```python
from build123d import *

# Parameters (mm, degrees)
BOSS_EXTRUDE1_DEPTH = 12
BOSS_EXTRUDE2_DEPTH = 15
SKETCH3_R           = 5
BOSS_EXTRUDE3_DEPTH = 25
CHAMFER1_SIZE       = 0.5


with BuildPart() as part:
    # Sketch1 → Boss-Extrude1 (new body)
    with BuildSketch(Plane.XY):
        with BuildLine():
            Line((2.645751311, 3), (-2.645751311, 3))
            ThreePointArc((-2.645751311, 3), (-1.645751311, -3.645751311), (4, 0))
            ThreePointArc((4, 0), (3.645751311, 1.645751311), (2.645751311, 3))
        make_face()
    extrude(amount=-BOSS_EXTRUDE1_DEPTH)

    # Sketch2 → Boss-Extrude2 (add)
    # profile 1 of 2: a face of its own
    with BuildSketch(Plane(origin=(0, 0, -12), x_dir=(-1, 0, 0), z_dir=(0, 0, -1))):
        with BuildLine():
            Line((5.656854249, 7), (-5.656854249, 7))
            ThreePointArc((-5.656854249, 7), (-9, 0), (-5.656854249, -7))
            Line((-5.656854249, -7), (5.656854249, -7))
            ThreePointArc((5.656854249, -7), (8.121320344, -3.878679656), (9, 0))
            ThreePointArc((9, 0), (8.121320344, 3.878679656), (5.656854249, 7))
        make_face()
        with BuildLine():
            ThreePointArc((2.645751311, 3), (0, -4), (-2.645751311, 3))
            Line((-2.645751311, 3), (2.645751311, 3))
        make_face(mode=Mode.SUBTRACT)
    # profile 2 of 2: a face of its own
    with BuildSketch(Plane(origin=(0, 0, -12), x_dir=(-1, 0, 0), z_dir=(0, 0, -1))):
        with BuildLine():
            Line((2.645751311, 3), (-2.645751311, 3))
            ThreePointArc((-2.645751311, 3), (0, -4), (2.645751311, 3))
        make_face()
    extrude(amount=BOSS_EXTRUDE2_DEPTH)

    # Sketch3 → Boss-Extrude3 (add)
    with BuildSketch(Plane(origin=(0, 0, -27), x_dir=(-1, 0, 0), z_dir=(0, 0, -1))):
        Circle(SKETCH3_R)
    extrude(amount=BOSS_EXTRUDE3_DEPTH)

    # Chamfer1
    chamfer1_edges = [part.edges().sort_by_distance(p)[0] for p in [
        (5, 0, -52),
        (0, 3, 0),
        (0, -4, 0),
    ]]
    chamfer(chamfer1_edges, length=CHAMFER1_SIZE)


solid = part.part
```
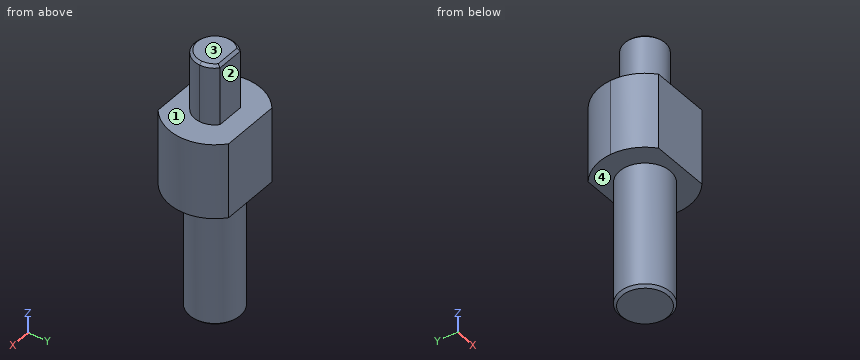
Could you check a few things on this model? Use its own coordinates, in mm. Face numbers are marked on the shaded views. A direction names the side the tool comes from. Round coordinates to 2 decimals unless told otherwise and drop trailing zeros. Loops run counter-clockwise (first coordinate to the right, second up) from the corner with the lowest first, then second, coordinate; pieces in that order, holes last. Notation, with made-up numbers: (59, 78) - (108, 78) arc R13 ccw to (108, 91) - close; hole circle Ø9 at (-19.5, 42). An arc over 180 degrees is marked (long way). Answer in a Markdown table with one row per item. Add a question column.
(1) If we section it at A-A (x = 0): Please give me the cut outline in (y, z), plus the area to 4 significant figures.
(2) If we section it at B-B (z = -7): Please give me the cut outline in (x, y).
(3) If we section it at C-C (z = -19): Please give me the cut outline in (x, y).
(4) For the marked faces 1, 2, 3 and 4, which set-ups out of +Z, -Z, +X, -X, +Y, -Y let a thin tool reach every point of the face, with its end or its side?
(5) I need wall thicknesses on line 1 along Z through (x, y) = (-4.75, -3.5); line 2 along Y through (x, z) = (-0.25, -35); line 3 along X through (y, z) = (-4, -14.5). Which ranges of each line are inside material? Lowest first, please.
(6) If we section it at D-D (y = -5.75): Please give me the cut outline in (x, z).
(7) I'm going to push flat-ended pins straight in: pin 1 (6 mm diameter, centred on y = -5, z = -24, fed in from -X); pin 2 (5 mm diameter, centred on x = 1.5, z = -44.5, fed in from +Y); pin 3 (3 mm diameter, centred on x = -7, y = -5.5, fed in from +Z). Where does each tip first touch, or does it pass through?
Model answer:
| question | item | result |
|---|---|---|
| 1 | outline | (-7, -27) - (-5, -27) - (-5, -51.5) - (-4.5, -52) - (4.5, -52) - (5, -51.5) - (5, -27) - (7, -27) - (7, -12) - (3, -12) - (3, -0.5) - (2.5, 0) - (-3.5, 0) - (-4, -0.5) - (-4, -12) - (-7, -12) - close |
| 1 | area | 543.5 mm² |
| 2 | outline | (-2.65, 3) arc R4 ccw (long way) to (2.65, 3) - close |
| 3 | outline | (-5.66, -7) - (5.66, -7) arc R9 ccw to (5.66, 7) - (-5.66, 7) arc R9 ccw to start |
| 4 | face 1 | +Z |
| 4 | face 2 | +Z, +X, -X, +Y |
| 4 | face 3 | +Z, +X, -X, +Y, -Y |
| 4 | face 4 | -Z |
| 5 | line 1 | z = -27 to -12 |
| 5 | line 2 | y = -4.99 to 4.99 |
| 5 | line 3 | x = -8.06 to 8.06 |
| 6 | outline | (-6.92, -27) - (6.92, -27) - (6.92, -12) - (-6.92, -12) - close |
| 7 | pin 1 | stops at x = -8.77 |
| 7 | pin 2 | stops at y = 5 |
| 7 | pin 3 | stops at z = -12 |
